from build123d import *

# Parameters (mm, degrees)
SKETCH1_W                   = 43.5
SKETCH1_H                   = 43.5
SKETCH1_W_2                 = 40.5
SKETCH1_H_2                 = 40.5
BOSS_EXTRUDE1_DEPTH         = 300
SKETCH2_W                   = 43.5
SKETCH2_H                   = 43.5
BOSS_EXTRUDE2_DEPTH         = 30
M8_TAPPED_HOLE1_D           = 6.8
M8_TAPPED_HOLE1_CSINK_D     = 8.05
M8_TAPPED_HOLE1_CSINK_ANGLE = 90
CUT_EXTRUDE1_DEPTH          = 307.033086447
SKETCH6_R                   = 5
CUT_EXTRUDE2_DEPTH          = 306.823478497


with BuildPart() as part:
    # Sketch1 → Boss-Extrude1 (new body)
    with BuildSketch(Plane.XY):
        with Locations((-20.25, 20.25)):
            Rectangle(SKETCH1_W, SKETCH1_H)
        with Locations((-20.25, 20.25)):
            Rectangle(SKETCH1_W_2, SKETCH1_H_2, mode=Mode.SUBTRACT)
    extrude(amount=BOSS_EXTRUDE1_DEPTH)

    # Sketch2 → Boss-Extrude2 (add)
    with BuildSketch(Plane(origin=(0, 0, 0), x_dir=(-1, 0, 0), z_dir=(0, 0, -1))):
        with Locations((20.25, 20.25)):
            Rectangle(SKETCH2_W, SKETCH2_H)
    extrude(amount=-BOSS_EXTRUDE2_DEPTH)

    # M8 Tapped Hole1 (through all)
    with Locations(Plane(origin=(0, 42, 0), x_dir=(1, 0, 0), z_dir=(0, 1, 0))):
        with Locations((-20.25, -220), (-20.25, -80)):
            CounterSinkHole(M8_TAPPED_HOLE1_D / 2, M8_TAPPED_HOLE1_CSINK_D / 2, counter_sink_angle=M8_TAPPED_HOLE1_CSINK_ANGLE)

    # Sketch5 → Cut-Extrude1 (cut, through all)
    with BuildSketch(Plane(origin=(0, 42, 0), x_dir=(1, 0, 0), z_dir=(0, 1, 0))):
        with BuildLine():
            Line((-35.25, 0), (-5.25, 0))
            ThreePointArc((-5.25, 0), (-20.25, -15), (-35.25, 0))
        make_face()
    extrude(amount=-CUT_EXTRUDE1_DEPTH, mode=Mode.SUBTRACT)

    # Sketch6 → Cut-Extrude2 (cut, through all)
    with BuildSketch(Plane(origin=(0, 0, 0), x_dir=(-1, 0, 0), z_dir=(0, 0, -1))):
        with Locations((20.25, 20.25)):
            Circle(SKETCH6_R)
    extrude(amount=-CUT_EXTRUDE2_DEPTH, mode=Mode.SUBTRACT)


solid = part.part
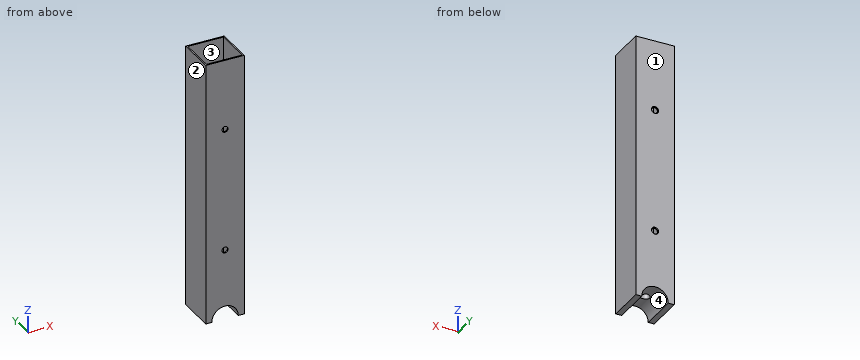
Work out the finished part from the listing and answer in its coordinate system (mm). Face numbers are marked on the shaded views. Round coordinates to 2 decimals unless told otherwise and drop trailing zeros. Write each loop counter-clockwise with the first axis right and the second up, starting at its lowest first coordinate (ties: lowest second). Pieces come first, ordered by that corner, then holes. Notation, with made-up numbers: (-39.75, 62.25) -> (-1.75, 62.25) arc R15 cw to (-1.75, 83.25) -> close; hole circle Ø4 at (-0.75, 20.5). An arc over 180 degrees is marked (long way). Answer as CSV lines item,"result". Start each with the question number.
(1) The part is cut by section D-D, the plane z = 35. Give the vertices of the cut face in (x, y), then the cut area to 3 significant figures.
(2) Each of these flat-tipped pins is pushed along its axis until it touches: pin 1 (6 mm diameter, centred on x = -9.5, y = 36, fed in from -Z); pin 2 (4 mm diameter, centred on x = -20.25, z = 220, fed in from -Y); pin 3 (12 mm diameter, centred on x = -8, y = 12.5, fed in from +Z); pin 4 (16 mm diameter, centred on x = -20.25, y = 20.25, fed in from -Z). Where does it stop, or does it pass through?
(3) The part is cut by section C-C, the plane y = 5.5. Give the vertices of the cut face in (x, z), then the cut area to 3 significant figures.
(4) The part is cut by section B-B, the plane y = 20.25. Give the vertices of the cut face in (x, z).
(5) The mould has two halves that part along X. Classify the marked faces 1, 2, 3 and 4: +X half, -X half, draft (parallel to the pull), parting line (faces both ways), or undercut.
(6) Find the intervals of material crossed by probe 1 along Z at (x, y) = (-20, 41); probe 2 along X at (y, z) = (24.5, 154.5); probe 3 along Y at (x, z) = (-3.5, 172), in increasing order.
(7) The part is cut by section A-A, the plane z = 80. Give the vertices of the cut face in (x, y) (3 decimals), then the cut area to 3 significant figures.
Output values:
1,outline,"(-42, -1.5) -> (1.5, -1.5) -> (1.5, 42) -> (-42, 42) -> close; hole (-40.5, 0) -> (0, 0) -> (0, 40.5) -> (-40.5, 40.5) -> close"
1,area,"252 mm²"
2,pin 1,"stops at z = 5.99"
2,pin 2,"passes through"
2,pin 3,"stops at z = 30"
2,pin 4,"stops at z = 12.69"
3,outline,"(-42, 0) -> (-35.25, 0) arc R15 cw to (-5.25, 0) -> (1.5, 0) -> (1.5, 300) -> (0, 300) -> (0, 30) -> (-40.5, 30) -> (-40.5, 300) -> (-42, 300) -> close"
3,area,"1,760 mm²"
4,outline,"(-42, 0) -> (-35.25, 0) arc R15 cw to (-25.25, 14.14) -> (-25.25, 30) -> (-40.5, 30) -> (-40.5, 300) -> (-42, 300) -> close; (-15.25, 14.14) arc R15 cw to (-5.25, 0) -> (1.5, 0) -> (1.5, 300) -> (0, 300) -> (0, 30) -> (-15.25, 30) -> close"
5,face 1,"draft"
5,face 2,"-X half"
5,face 3,"undercut"
5,face 4,"undercut"
6,probe 1,"z = 15 to 76.61, 83.39 to 216.61, 223.39 to 300"
6,probe 2,"x = -42 to -40.5, 0 to 1.5"
6,probe 3,"y = -1.5 to 0, 40.5 to 42"
7,outline,"(-42, -1.5) -> (-23.65, -1.5) -> (-23.65, 0) -> (-40.5, 0) -> (-40.5, 40.5) -> (-23.65, 40.5) -> (-23.65, 41.375) -> (-24.275, 42) -> (-42, 42) -> close; (-16.85, -1.5) -> (1.5, -1.5) -> (1.5, 42) -> (-16.225, 42) -> (-16.85, 41.375) -> (-16.85, 40.5) -> (0, 40.5) -> (0, 0) -> (-16.85, 0) -> close"
7,area,"231 mm²"
